Could you check a few things on this model? Use its own coordinates, in mm. A direction names the side the tool comes from. Give positions to 0.01 mm unless a question says otherwise; leave off trailing zeros. Loops run counter-clockwise (first coordinate to the right, second up) from the corner with the lowest first, then second, coordinate; pieces in that order, holes last. Notation, with made-up numbers: (6.25, 49.25) -> (37.25, 49.25) arc R15 cw to (37.25, 71.25) -> close; hole circle Ø9 at (83.5, 32.5). An arc over 180 degrees is marked (long way). Put each result on its own line as item: value.
```python
from build123d import *

# Parameters (mm, degrees)
SKETCH1_W                                         = 120
SKETCH1_H                                         = 200
EXTRUDE1_DEPTH                                    = 6
SKETCH3_W                                         = 19
SKETCH3_H                                         = 152
CUT_EXTRUDE1_DEPTH                                = 118.234807118
FILLET1_R                                         = 5
SKETCH4_W                                         = 20
SKETCH4_H                                         = 45
CUT_EXTRUDE2_DEPTH                                = 118.234807118
SKETCH6_R                                         = 2.5
CUT_EXTRUDE3_DEPTH                                = 118.234807118
M5_SOCKET_HEAD_CAP_SCREW_COUNTERBORE1_D           = 5.5
M5_SOCKET_HEAD_CAP_SCREW_COUNTERBORE1_CBORE_D     = 10
M5_SOCKET_HEAD_CAP_SCREW_COUNTERBORE1_CBORE_DEPTH = 6
M5_TAPPED_HOLE1_D                                 = 4.2
FILLET2_R                                         = 5
M5_TAPPED_HOLE2_D                                 = 4.2
M5_TAPPED_HOLE2_DEPTH                             = 12.4
M5_TAPPED_HOLE2_TIP                               = 1.2618073
M5_TAPPED_HOLE3_D                                 = 4.2


with BuildPart() as part:
    # Sketch1 → Extrude1 (new, symmetric)
    with BuildSketch(Plane(origin=(0, 0, 0), x_dir=(1, 0, 0), z_dir=(0, 1, 0))):
        Rectangle(SKETCH1_W, SKETCH1_H)
    extrude(amount=EXTRUDE1_DEPTH, both=True)

    # Sketch3 → Cut-Extrude1 (cut, through all)
    with BuildSketch(Plane(origin=(0, 6, 0), x_dir=(1, 0, 0), z_dir=(0, 1, 0))):
        with Locations((-50.5, -24)):
            Rectangle(SKETCH3_W, SKETCH3_H)
    extrude(amount=-CUT_EXTRUDE1_DEPTH, mode=Mode.SUBTRACT)

    # Fillet1
    fillet1_edges = [part.edges().sort_by_distance(p)[0] for p in [
        (-41, 0, -52),
    ]]
    fillet(fillet1_edges, radius=FILLET1_R)

    # Sketch4 → Cut-Extrude2 (cut, through all)
    with BuildSketch(Plane(origin=(0, 6, 0), x_dir=(1, 0, 0), z_dir=(0, 1, 0))):
        with Locations((50, -77.5)):
            Rectangle(SKETCH4_W, SKETCH4_H)
    extrude(amount=-CUT_EXTRUDE2_DEPTH, mode=Mode.SUBTRACT)

    # Sketch6 → Cut-Extrude3 (cut, through all)
    with BuildSketch(Plane(origin=(0, 6, 0), x_dir=(1, 0, 0), z_dir=(0, 1, 0))):
        with Locations(Location((12.5, 40, 0), (0, 0, 270))):
            Circle(SKETCH6_R)
        with Locations(Location((12.5, -40, 0), (0, 0, 270))):
            Circle(SKETCH6_R)
    extrude(amount=-CUT_EXTRUDE3_DEPTH, mode=Mode.SUBTRACT)

    # M5 Socket Head Cap Screw Counterbore1 (through all)
    with Locations(Plane(origin=(37.5, 6, -40), x_dir=(0, 0, 1), z_dir=(0, 1, 0))):
        with Locations((0, 0), (0, -50), (80, -50), (80, 0)):
            CounterBoreHole(M5_SOCKET_HEAD_CAP_SCREW_COUNTERBORE1_D / 2, M5_SOCKET_HEAD_CAP_SCREW_COUNTERBORE1_CBORE_D / 2, M5_SOCKET_HEAD_CAP_SCREW_COUNTERBORE1_CBORE_DEPTH)

    # M5 Tapped Hole1 (through all)
    with Locations(Plane(origin=(32, 6, 85), x_dir=(0, 0, 1), z_dir=(0, 1, 0))):
        with Locations((0, 0), (0, -65), (-150, 0), (-150, -65)):
            Hole(M5_TAPPED_HOLE1_D / 2)

    # Fillet2
    fillet2_edges = [part.edges().sort_by_distance(p)[0] for p in [
        (40, 0, 55),
    ]]
    fillet(fillet2_edges, radius=FILLET2_R)

    # M5 Tapped Hole2
    with Locations(Plane(origin=(40, 0, 91), x_dir=(0, 0, 1), z_dir=(1, 0, 0))):
        with Locations((0, 0), (-20, 0)):
            Hole(M5_TAPPED_HOLE2_D / 2, depth=M5_TAPPED_HOLE2_DEPTH)
            with Locations((0, 0, -(M5_TAPPED_HOLE2_DEPTH + M5_TAPPED_HOLE2_TIP / 2))):  # 118° drill point
                Cone(0, M5_TAPPED_HOLE2_D / 2, M5_TAPPED_HOLE2_TIP, mode=Mode.SUBTRACT)

    # M5 Tapped Hole3 (through all)
    with Locations(Plane(origin=(50, 6, -40), x_dir=(0, 0, 1), z_dir=(0, 1, 0))):
        with Locations((0, 0), (80, 0)):
            Hole(M5_TAPPED_HOLE3_D / 2)


solid = part.part
```
1. If we section it at A-A (x = 37.5): List the corners of the cut face in (y, z) for me.
Recorded:
outline: (-6, -100) -> (6, -100) -> (6, -45) -> (0, -45) -> (0, -42.75) -> (-6, -42.75) -> close; (-6, -37.25) -> (0, -37.25) -> (0, -35) -> (6, -35) -> (6, 35) -> (0, 35) -> (0, 37.25) -> (-6, 37.25) -> close; (-6, 42.75) -> (0, 42.75) -> (0, 45) -> (6, 45) -> (6, 100) -> (-6, 100) -> close; hole circle Ø4.2 at (0, 71); hole circle Ø4.2 at (0, 91)
2. If we section it at C-C (x = -12.5): List the corners of the cut face in (y, z) for me.
Recorded:
outline: (-6, -100) -> (6, -100) -> (6, -45) -> (0, -45) -> (0, -42.75) -> (-6, -42.75) -> close; (-6, -37.25) -> (0, -37.25) -> (0, -35) -> (6, -35) -> (6, 35) -> (0, 35) -> (0, 37.25) -> (-6, 37.25) -> close; (-6, 42.75) -> (0, 42.75) -> (0, 45) -> (6, 45) -> (6, 100) -> (-6, 100) -> close
3. I need wall thicknesses on line 1 (X direction, y = 2, z = -40); line 2 (X direction, y = -2, z = -40); line 3 (Z direction, x = -15.5, y = 3). Which ranges of each line are inside material? Lowest first, please.
Recorded:
line 1: x = -41 to -17.5, -7.5 to 10, 15 to 32.5, 42.5 to 47.9, 52.1 to 60
line 2: x = -41 to -15.25, -9.75 to 10, 15 to 34.75, 40.25 to 47.9, 52.1 to 60
line 3: z = -100 to -44, -36 to 36, 44 to 100
4. If we section it at D-D (z = -40): List the corners of the cut face in (x, y) for me, then the cut area to 3 significant figures.
Recorded:
outline: (-41, -6) -> (-15.25, -6) -> (-15.25, 0) -> (-17.5, 0) -> (-17.5, 6) -> (-41, 6) -> close; (-9.75, -6) -> (10, -6) -> (10, 6) -> (-7.5, 6) -> (-7.5, 0) -> (-9.75, 0) -> close; (15, -6) -> (34.75, -6) -> (34.75, 0) -> (32.5, 0) -> (32.5, 6) -> (15, 6) -> close; (40.25, -6) -> (47.9, -6) -> (47.9, 6) -> (42.5, 6) -> (42.5, 0) -> (40.25, 0) -> close; (52.1, -6) -> (60, -6) -> (60, 6) -> (52.1, 6) -> close
area: 916 mm^2
5. I'm going to push flat-ended pins straight in: pin 1 (4 mm diameter, centred on y = 0, z = 91, fed in from +X); pin 2 (4 mm diameter, centred on x = -33, z = -65, fed in from -Y); pin 3 (5 mm diameter, centred on y = 4, z = 23, fed in from -X); pin 4 (1 mm diameter, centred on x = -45.5, y = 4, fed in from +Z). Where does each tip first touch, or does it pass through?
Recorded:
pin 1: stops at x = 27.54
pin 2: passes through
pin 3: stops at x = -41
pin 4: stops at z = -51.9
6. For faces 1 (the face through (-41, 0, 28)), 2 (the face through (35, 0, 42)), 3 (the face through (33.71, -0.09, 93.1)), which set-ups out of +Z, -Z, +X, -X, +Y, -Y let a thin tool reach every point of the face, with its end or its side?
Recorded:
face 1: +Z, -X, +Y, -Y
face 2: +Y
face 3: +X
7. Thinking about a two-plate mould opening in Z: for faces 4 (the face through (-43, 0, -51)), 5 (the face through (-1, 6, -1)), 6 (the face through (26.56, 0.14, 71.34)), which applies, pulls with the +Z half, pulls with the -Z half, needs draft (parallel to the pull), parting line crosses it, or undercut?
Recorded:
face 4: pulls with the +Z half
face 5: needs draft
face 6: undercut
8. If we section it at B-B (z = 85): List the corners of the cut face in (x, y) for me.
Recorded:
outline: (-41, -6) -> (-35.1, -6) -> (-35.1, 6) -> (-41, 6) -> close; (-30.9, -6) -> (29.9, -6) -> (29.9, 6) -> (-30.9, 6) -> close; (34.1, -6) -> (40, -6) -> (40, 6) -> (34.1, 6) -> close
